Can you work these out from the model? Positions are in its coordinate system, mm. Face numbers are marked on the shaded views. A direction names the side the tool comes from. Round coordinates to 2 decimals unless told otherwise and drop trailing zeros. Write each loop counter-clockwise with the first axis right and the second up, starting at its lowest first coordinate (ties: lowest second). Pieces come first, ordered by that corner, then holes.
Q1. I'm going to push flat-ended pins straight in: pin 1 Ø13 at (y, z) = (11, 343) entering from -X; pin 2 Ø1 at (x, z) = (2, 90) entering from -Y; pin 3 Ø5 at (y, z) = (5.5, -303.5) entering from -X. Where does each tip first touch, or does it pass through?
Q2. If we section it at D-D (x = 325): Please give me the cut outline in (y, z).
Q3. If we section it at C-C (y = -10): Please give me the cut outline in (x, z).
Q4. For the marked faces 1 and 2, which set-ups out of +Z, -Z, +X, -X, +Y, -Y let a thin tool reach every point of the face, with its end or its side?
Q5. If we section it at A-A (x = 129): Please give me the cut outline in (y, z).
Q6. Please list where these lines run through material, in increasing order: line 1 along Y through (x, z) = (300.5, 236); line 2 along X through (y, z) = (-39.5, -167.5); line 3 along X through (y, z) = (-97.5, 150).
Q7. If we section it at B-B (z = 238.5): Please give me the cut outline in (x, y), plus the area to 3 significant figures.
from build123d import *

# Parameters (mm, degrees)
BOSS_EXTRUDE1_DEPTH     = 348
CUT_EXTRUDE1_DEPTH      = 554.754458221
CUT_EXTRUDE1_DEPTH_BACK = 554.754458221
CUT_EXTRUDE3_DEPTH      = 717.846566568


with BuildPart() as part:
    # Sketch1 → Boss-Extrude1 (new, symmetric)
    with BuildSketch(Plane.XY):
        with BuildLine():
            Line((0, 0), (418, 0))
            Line((418, 0), (418, 9))
            Line((418, 9), (403, 16))
            Line((403, 16), (0, 16))
            ThreePointArc((0, 16), (-88.953996871, -17.784300428), (-133.053537704, -102.101694915))
            Line((-133.053537704, -102.101694915), (-117.166548127, -104))
            ThreePointArc((-117.166548127, -104), (-78.33262411, -29.750354108), (0, 0))
        make_face()
    extrude(amount=BOSS_EXTRUDE1_DEPTH, both=True)

    # Sketch2 → Cut-Extrude1 (cut, two sides: drawn at the far end of the back side and taken through both)
    with BuildSketch(Plane(origin=(0, 0, 0), x_dir=(1, 0, 0), z_dir=(0, 1, 0)).offset(-CUT_EXTRUDE1_DEPTH_BACK)):
        with BuildLine():
            Line((86, -256), (86, -230))
            ThreePointArc((86, -230), (84.535533906, -226.464466094), (81, -225))
            Line((81, -225), (-133.053537704, -225))
            Line((-133.053537704, -225), (-133.053537704, -348))
            Line((-133.053537704, -348), (86, -348))
            Line((86, -348), (86, -332))
            ThreePointArc((86, -332), (88.928932188, -324.928932188), (96, -322))
            Line((96, -322), (141, -322))
            ThreePointArc((141, -322), (144.535533906, -320.535533906), (146, -317))
            Line((146, -317), (146, -271))
            ThreePointArc((146, -271), (144.535533906, -267.464466094), (141, -266))
            Line((141, -266), (96, -266))
            ThreePointArc((96, -266), (88.928932188, -263.071067812), (86, -256))
        make_face()
        with BuildLine():
            Line((96, 322), (141, 322))
            ThreePointArc((141, 322), (144.535533906, 320.535533906), (146, 317))
            Line((146, 317), (146, 271))
            ThreePointArc((146, 271), (144.535533906, 267.464466094), (141, 266))
            Line((141, 266), (96, 266))
            ThreePointArc((96, 266), (88.928932188, 263.071067812), (86, 256))
            Line((86, 256), (86, 230))
            ThreePointArc((86, 230), (84.535533906, 226.464466094), (81, 225))
            Line((81, 225), (-133.053537704, 225))
            Line((-133.053537704, 225), (-133.053537704, 348))
            Line((-133.053537704, 348), (86, 348))
            Line((86, 348), (86, 332))
            ThreePointArc((86, 332), (88.928932188, 324.928932188), (96, 322))
        make_face()
    extrude(amount=CUT_EXTRUDE1_DEPTH + CUT_EXTRUDE1_DEPTH_BACK, mode=Mode.SUBTRACT)

    # Sketch3 → Cut-Extrude3 (cut, through all)
    with BuildSketch(Plane.XY.offset(225)):
        with BuildLine():
            Line((-120.305667655, -103.624912792), (-133.053537704, -102.101694915))
            ThreePointArc((-133.053537704, -102.101694915), (-127.139944881, -75.674659886), (-116.033703785, -50.976275946))
            ThreePointArc((-116.033703785, -50.976275946), (-120.754032763, -62.041779759), (-122.694651189, -73.9144745))
            ThreePointArc((-122.694651189, -73.9144745), (-122.404927497, -88.842445048), (-120.305667655, -103.624912792))
        make_face()
    extrude(amount=-CUT_EXTRUDE3_DEPTH, mode=Mode.SUBTRACT)


solid = part.part
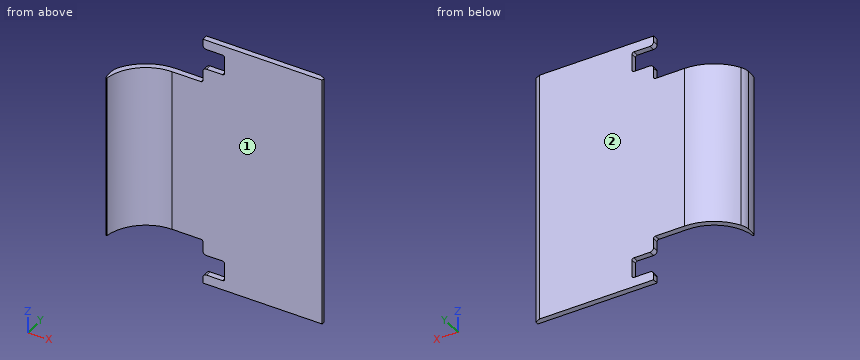
A:
1. pin 1: stops at x = 86
1. pin 2: stops at y = 0
1. pin 3: stops at x = 146
2. outline: (0, -348) - (16, -348) - (16, 348) - (0, 348) - close
3. outline: (-79.32, -225) - (-47.54, -225) - (-47.54, 225) - (-79.32, 225) - close
4. face 1: +Z, -Z, +X, -Y
4. face 2: +Z, -Z, +X, -X, +Y
5. outline: (0, -348) - (16, -348) - (16, -322) - (0, -322) - close; (0, -266) - (16, -266) - (16, 266) - (0, 266) - close; (0, 322) - (16, 322) - (16, 348) - (0, 348) - close
6. line 1: y = 0 to 16
6. line 2: x = -108.6 to -88.1
6. line 3: x = -121.4 to -116.21
7. outline: (86, 0) - (418, 0) - (418, 9) - (403, 16) - (86, 16) - close
7. area: 5,260 mm2
